Geometry: final body of the model. Coordinates: model frame, mm. Round coordinates to 2 decimals unless told otherwise and drop trailing zeros. Write each loop counter-clockwise with the first axis right and the second up, starting at its lowest first coordinate (ties: lowest second). Pieces come first, ordered by that corner, then holes.
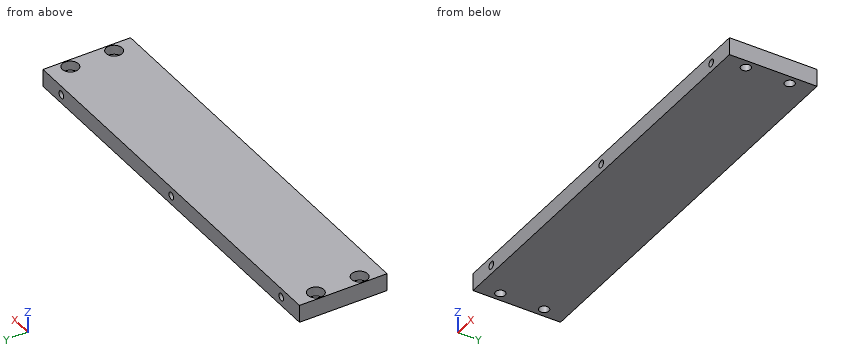
from build123d import *

# Parameters (mm, degrees)
SKETCH_1_W                     = 280
SKETCH_1_H                     = 60
EXTRUDE_1_DEPTH                = 12
HOLE_WIZARD_M6_1_D             = 5
HOLE_WIZARD_M6_1_DEPTH         = 15
HOLE_WIZARD_M6_1_TIP           = 1.502151548
HOLE_WIZARD_M6_2_D             = 5
HOLE_WIZARD_M6_2_DEPTH         = 15
HOLE_WIZARD_M6_2_TIP           = 1.502151548
HOLE_WIZARD_M6_1_2_D           = 6.6
HOLE_WIZARD_M6_1_2_CBORE_D     = 11
HOLE_WIZARD_M6_1_2_CBORE_DEPTH = 6.4


with BuildPart() as part:
    # 草图1 → 凸台-拉伸1 (new body)
    with BuildSketch(Plane.XY):
        with Locations((140, -30)):
            Rectangle(SKETCH_1_W, SKETCH_1_H)
    extrude(amount=EXTRUDE_1_DEPTH)

    # Hole Wizard M6 _1
    with Locations(Plane(origin=(0, 0, 0), x_dir=(1, 0, 0), z_dir=(0, 1, 0))):
        with Locations((260, -6), (140, -6), (20, -6)):
            Hole(HOLE_WIZARD_M6_1_D / 2, depth=HOLE_WIZARD_M6_1_DEPTH)
            with Locations((0, 0, -(HOLE_WIZARD_M6_1_DEPTH + HOLE_WIZARD_M6_1_TIP / 2))):  # 118° drill point
                Cone(0, HOLE_WIZARD_M6_1_D / 2, HOLE_WIZARD_M6_1_TIP, mode=Mode.SUBTRACT)

    # M6 螺纹孔2
    with Locations(Plane(origin=(0, -60, 0), x_dir=(-1, 0, 0), z_dir=(0, -1, 0))):
        with Locations((-260, -6), (-140, -6), (-20, -6)):
            Hole(HOLE_WIZARD_M6_2_D / 2, depth=HOLE_WIZARD_M6_2_DEPTH)
            with Locations((0, 0, -(HOLE_WIZARD_M6_2_DEPTH + HOLE_WIZARD_M6_2_TIP / 2))):  # 118° drill point
                Cone(0, HOLE_WIZARD_M6_2_D / 2, HOLE_WIZARD_M6_2_TIP, mode=Mode.SUBTRACT)

    # Hole Wizard M6 _1 2 (through all)
    with Locations(Plane.XY.offset(12)):
        with Locations((274, -45), (274, -15), (6, -45), (6, -15)):
            CounterBoreHole(HOLE_WIZARD_M6_1_2_D / 2, HOLE_WIZARD_M6_1_2_CBORE_D / 2, HOLE_WIZARD_M6_1_2_CBORE_DEPTH)


solid = part.part
1) Section A-A on x = 274. Output: boundary loops of the cut face in (y, z).
2) Line query: probe 1 along X at (y, z) = (-44.5, 0.5); probe 2 along Y at (x, z) = (6, 8); probe 3 along Y at (x, z) = (274, 2). Output: solid intervals per line, ascending.
3) First-contact query: P1, Ø6, axis at y = -27, z = 5.5, coming from the -X side; P2, Ø4.5, axis at x = 260, z = 6, coming from the +Y side; P3, Ø4, axis at x = 6, y = -15, coming from the -Z side; P4, Ø9, axis at x = 6, y = -45, coming from the +Z side. Flat tips, straight axial feed; report the tip coordinate or a pass-through.
Filled in:
1. outline: (-60, 0) - (-48.3, 0) - (-48.3, 5.6) - (-50.5, 5.6) - (-50.5, 12) - (-60, 12) - close; (-41.7, 0) - (-18.3, 0) - (-18.3, 5.6) - (-20.5, 5.6) - (-20.5, 12) - (-39.5, 12) - (-39.5, 5.6) - (-41.7, 5.6) - close; (-11.7, 0) - (0, 0) - (0, 12) - (-9.5, 12) - (-9.5, 5.6) - (-11.7, 5.6) - close
2. probe 1: x = 0 to 2.74, 9.26 to 270.74, 277.26 to 280
2. probe 2: y = -60 to -50.5, -39.5 to -20.5, -9.5 to 0
2. probe 3: y = -60 to -48.3, -41.7 to -18.3, -11.7 to 0
3. P1: stops at x = 0
3. P2: stops at y = -15.15
3. P3: passes through
3. P4: stops at z = 5.6
